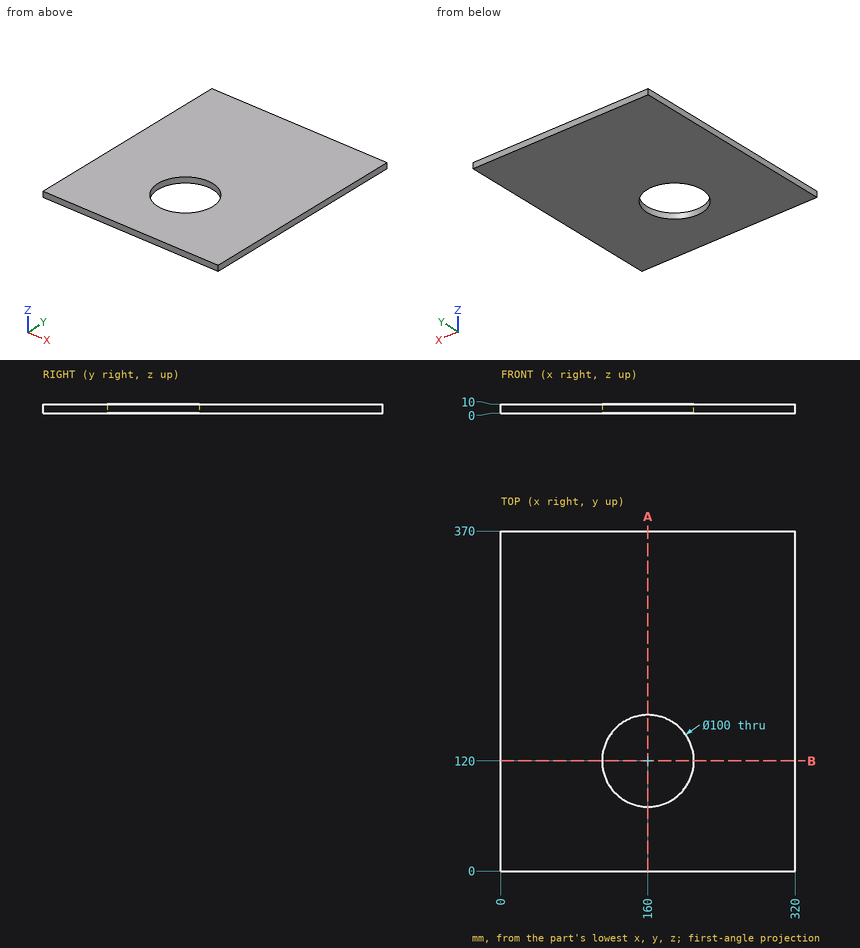
Job drawing, mm, ordinate dimensions from the low corner. One solid piece. Give positions to 0.01 mm unless a question says otherwise; leave off trailing zeros. Order: outer loops, then holes, each group sorted by start corner. A loop starts at its lowest first (then second) coordinate and runs counter-clockwise, first axis right, second up. Notation, with made-up numbers: (52.25, 15.5) -> (77.25, 15.5) arc R16 cw to (77.25, 34.5) -> close; hole circle Ø7 at (1.5, 57). An arc over 180 degrees is marked (long way). Return JSON: item names as keys, results as strings.
Q1. Saw through at B-B (y = 120). Write the cut outline in (x, z).
Working result:
{"outline": "(0, 0) -> (110, 0) -> (110, 10) -> (0, 10) -> close; (210, 0) -> (320, 0) -> (320, 10) -> (210, 10) -> close"}
Q2. Drill centre lines: line 1 (Y direction, x = 160, z = 4); line 2 (X direction, y = 87.5, z = 1.5); line 3 (Y direction, x = 197, z = 3.5). Where is each one in solid material? Low to high.
Working result:
{"line 1": "0 to 70, 170 to 370", "line 2": "0 to 122, 198 to 320", "line 3": "0 to 86.37, 153.63 to 370"}
Q3. Saw through at A-A (x = 160). Write the cut outline in (y, z), then the cut area to 3 significant figures.
Working result:
{"outline": "(0, 0) -> (70, 0) -> (70, 10) -> (0, 10) -> close; (170, 0) -> (370, 0) -> (370, 10) -> (170, 10) -> close", "area": "2,700 mm²"}
